Design review of the part built by this model. Coordinates are the model's own, in mm. Round coordinates to 2 decimals unless told otherwise and drop trailing zeros. Write each loop counter-clockwise with the first axis right and the second up, starting at its lowest first coordinate (ties: lowest second). Pieces come first, ordered by that corner, then holes. Notation, with made-up numbers: M 7,89.25 L 58,89.25 A36 ccw 58,126.25 Z; hole C 22.25,27.5 d7. An arc over 180 degrees is marked long. One line per question, with ' | ' between items. Start each with the question number.
Item 1: Insertion check: pin 1 Ø1 at (y, z) = (219.5, 1.5) entering from +X; pin 2 Ø1 at (x, z) = (55, 2.5) entering from -Y; pin 3 Ø2 at (x, z) = (-7, 6) entering from +Y. Each pin has a flat end and moves straight along its axis. Give the tip position at first contact, or say it passes through.
Item 2: Add section A-A, the plane y = 0. State the section outline as (x, z) points.
Item 3: Add section D-D, the plane y = -135.5. State the section outline as (x, z) points.
Item 4: Add section C-C, the plane x = 0. State the section outline as (y, z) points, and give its area (3 significant figures).
Item 5: Add section B-B, the plane z = 4.5. State the section outline as (x, y) points.
Item 6: For L1, parallel to Y at x = 0, z = 3.75; L2, parallel to Y at x = 9, z = 6; L3, parallel to X at y = -18, z = 10.75, list the stretches that pass through material, from the lowest coordinate up.
```python
from build123d import *

# Parameters (mm, degrees)
SKETCH1_R           = 30
BOSS_EXTRUDE1_DEPTH = 12


with BuildPart() as part:
    # Sketch1 → Boss-Extrude1 (new body)
    with BuildSketch(Plane.XY):
        with BuildLine():
            Line((-140, 247.683496575), (-140, -164.068744093))
            ThreePointArc((-140, -164.068744093), (-132.043654713, -179.006113339), (-115.208333333, -180.738275097))
            ThreePointArc((-115.208333333, -180.738275097), (-17.836743976, -126.110196806), (63.088864614, -49.191413496))
            ThreePointArc((63.088864614, -49.191413496), (79.995195531, 0.876750818), (61.995559096, 50.562344213))
            Line((61.995559096, 50.562344213), (-108.050999203, 259.060024023))
            ThreePointArc((-108.050999203, 259.060024023), (-128.038128256, 264.640530725), (-140, 247.683496575))
        make_face()
        Circle(SKETCH1_R, mode=Mode.SUBTRACT)
    extrude(amount=BOSS_EXTRUDE1_DEPTH)


solid = part.part
```
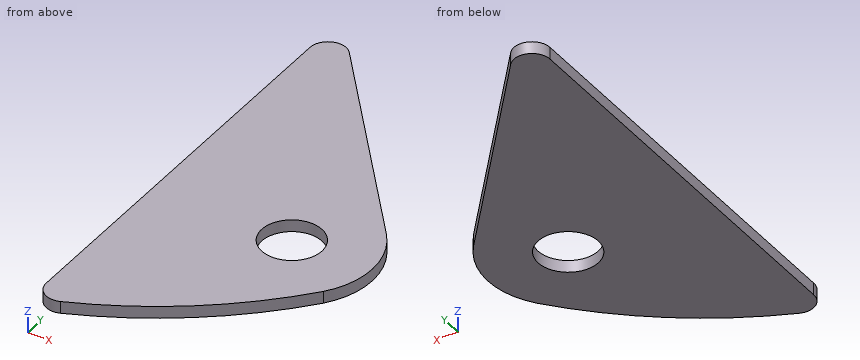
Computed values:
1) pin 1: stops at x = -75.38 | pin 2: stops at y = -59.36 | pin 3: stops at y = 136.39
2) outline: M -140,0 L -30,0 L -30,12 L -140,12 Z; M 30,0 L 80,0 L 80,12 L 30,12 Z
3) outline: M -140,0 L -31.06,0 L -31.06,12 L -140,12 Z
4) outline: M -112.25,0 L -30,0 L -30,12 L -112.25,12 Z; M 30,0 L 126.58,0 L 126.58,12 L 30,12 Z | area: 2,150 mm^2
5) outline: M -140,-164.07 A18 ccw -115.21,-180.74 A450 ccw 63.09,-49.19 A80 ccw 62,50.56 L -108.05,259.06 A18 ccw -140,247.68 Z; hole C 0,0 d60
6) L1: y = -112.25 to -30, 30 to 126.58 | L2: y = -104.68 to -28.62, 28.62 to 115.54 | L3: x = -140 to -24, 24 to 77.95
